Check sheet for the modelled part. Datum: model origin and axes. Units: mm. Face numbers are marked on the shaded views. A direction names the side the tool comes from. Round coordinates to 2 decimals unless told otherwise and drop trailing zeros. Order: outer loops, then holes, each group sorted by start corner. A loop starts at its lowest first (then second) coordinate and runs counter-clockwise, first axis right, second up. Notation, with made-up numbers: (38.5, -19.5) -> (49.5, -19.5) arc R17 ccw to (49.5, -8.5) -> close; hole circle Ø5 at (17, 22.5). An arc over 180 degrees is marked (long way). Answer in a Markdown table with one row per item.
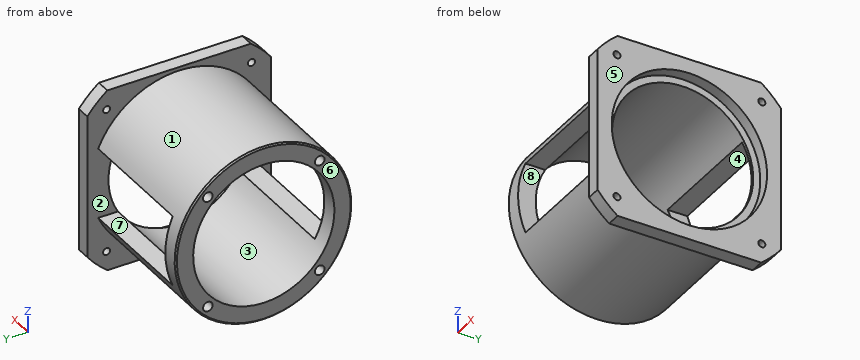
```python
from build123d import *

# Parameters (mm, degrees)
SKETCH_1_R               = 62.5
EXTRUDE_1_DEPTH          = 100
SKETCH_2_R               = 82.5
EXTRUDE_2_DEPTH          = 10
SKETCH_3_OUTSIDE_W       = 218.594
SKETCH_3_OUTSIDE_H       = 218.594
SKETCH_3_OUTSIDE_W_2     = 130
SKETCH_3_OUTSIDE_H_2     = 130
CUT_EXTRUDE_1_DEPTH      = 161.351177108
SKETCH_4_R               = 55
CUT_EXTRUDE_2_DEPTH      = 8
PATTERN_CIRCULAR_1_COUNT = 4
SKETCH_7_R               = 50
CUT_EXTRUDE_3_DEPTH      = 138.309868546
CUT_EXTRUDE_4_DEPTH      = 144.352711868
CUT_EXTRUDE_4_DEPTH_BACK = 144.352711868
SKETCH_8_W               = 88
SKETCH_8_H               = 50
PATTERN_CIRCULAR_2_COUNT = 4
CHAMFER_1_SIZE           = 1


with BuildPart() as part:
    # 草图1 → 凸台-拉伸1 (new body)
    with BuildSketch(Plane(origin=(0, 0, 0), x_dir=(0, 0, -1), z_dir=(1, 0, 0))):
        Circle(SKETCH_1_R)
    extrude(amount=EXTRUDE_1_DEPTH)

    # 草图2 → 凸台-拉伸2 (add)
    with BuildSketch(Plane(origin=(100, 0, 0), x_dir=(0, 0, -1), z_dir=(1, 0, 0))):
        Circle(SKETCH_2_R)
    extrude(amount=EXTRUDE_2_DEPTH)

    # 草图3 outside → 切除-拉伸1 (cut, through all)
    with BuildSketch(Plane(origin=(110, 0, 0), x_dir=(0, 0, -1), z_dir=(1, 0, 0))):
        Rectangle(SKETCH_3_OUTSIDE_W, SKETCH_3_OUTSIDE_H)
        Rectangle(SKETCH_3_OUTSIDE_W_2, SKETCH_3_OUTSIDE_H_2, mode=Mode.SUBTRACT)
    extrude(amount=-CUT_EXTRUDE_1_DEPTH, mode=Mode.SUBTRACT)

    # 草图4 → 切除-拉伸2 (cut)
    with BuildSketch(Plane(origin=(110, 0, 0), x_dir=(0, 0, -1), z_dir=(1, 0, 0))):
        Circle(SKETCH_4_R)
    extrude(amount=-CUT_EXTRUDE_2_DEPTH, mode=Mode.SUBTRACT)

    # 草图6 → M6 螺纹孔1 (revolve, cut)
    with BuildSketch(Plane(origin=(110, 51.265241636, 51.265241636), x_dir=(0, 0, -1), z_dir=(0, 1, 0))):
        Polygon((0, 0), (0, 16.502151548), (2.5, 15), (2.5, 0), align=None)
    hole_wizard_m6_1 = revolve(axis=Axis((116.35, 51.265241636, 51.265241636), (-1, 0, 0)), mode=Mode.SUBTRACT)

    # 阵列(圆周)1: M6 螺纹孔1 ×4 about axis
    pattern_circular_1_axis = Axis((0, 0, 0), (1, 0, 0))
    for i in range(1, PATTERN_CIRCULAR_1_COUNT):
        add(hole_wizard_m6_1.rotate(pattern_circular_1_axis, i * 360 / PATTERN_CIRCULAR_1_COUNT), mode=Mode.SUBTRACT)

    # 草图7 → 切除-拉伸3 (cut, through all)
    with BuildSketch(Plane(origin=(102, 0, 0), x_dir=(0, 0, -1), z_dir=(1, 0, 0))):
        Circle(SKETCH_7_R)
    extrude(amount=-CUT_EXTRUDE_3_DEPTH, mode=Mode.SUBTRACT)

    # 草图8 → 切除-拉伸4 (cut, two sides: drawn at the far end of the back side and taken through both)
    with BuildSketch(Plane(origin=(0, 0, 0), x_dir=(1, 0, 0), z_dir=(0, 1, 0)).offset(-CUT_EXTRUDE_4_DEPTH_BACK)):
        with Locations((56, 0)):
            Rectangle(SKETCH_8_W, SKETCH_8_H)
    extrude(amount=CUT_EXTRUDE_4_DEPTH + CUT_EXTRUDE_4_DEPTH_BACK, mode=Mode.SUBTRACT)

    # 草图10 → M8 螺纹孔1 (revolve, cut)
    with BuildSketch(Plane(origin=(0, 39.597979746, -39.597979746), x_dir=(0, 0, 1), z_dir=(0, 1, 0))):
        Polygon((0, 0), (0, 21.792926105), (3.4, 19.75), (3.4, 0), align=None)
    hole_wizard_m8_1 = revolve(axis=Axis((-6.35, 39.597979746, -39.597979746), (1, 0, 0)), mode=Mode.SUBTRACT)

    # 阵列(圆周)2: M8 螺纹孔1 ×4 about axis
    pattern_circular_2_axis = Axis((0, 0, 0), (1, 0, 0))
    for i in range(1, PATTERN_CIRCULAR_2_COUNT):
        add(hole_wizard_m8_1.rotate(pattern_circular_2_axis, i * 360 / PATTERN_CIRCULAR_2_COUNT), mode=Mode.SUBTRACT)

    # 倒角1
    chamfer_1_edges = [part.edges().sort_by_distance(p)[0] for p in [
        (0, 0, 62.5),
    ]]
    chamfer(chamfer_1_edges, length=CHAMFER_1_SIZE)


solid = part.part
```
(1) Tool access check on the marked faces 1, 2, 3 and 4. Record the directions out of +Z, -Z, +X, -X, +Y, -Y that give a thin tool (end or side, any length) a straight path to the whole face; none if there is none.
Solutions:
| item | result |
|---|---|
| face 1 | -X |
| face 2 | none |
| face 3 | +X, -X |
| face 4 | +Y, -Y |
(2) Draft check along X on the marked faces 5, 6, 7 and 8. Enter one of: pulls with the +X half, pulls with the -X half, needs draft (parallel to the pull), parting line crosses it, or undercut.
Solutions:
| item | result |
|---|---|
| face 5 | pulls with the +X half |
| face 6 | pulls with the -X half |
| face 7 | undercut |
| face 8 | undercut |
(3) Section check A-A on x = 50. Record the boundary of the cut face in (y, z), plus the area to 3 significant figures.
Solutions:
| item | result |
|---|---|
| outline | (-57.28, -25) arc R62.5 ccw to (57.28, -25) -> (43.3, -25) arc R50 cw to (-43.3, -25) -> close; (-57.28, 25) -> (-43.3, 25) arc R50 cw to (43.3, 25) -> (57.28, 25) arc R62.5 ccw to start |
| area | 3,120 mm^2 |
(4) Scan lines: probe 1 along Y at (x, z) = (103.5, -21); probe 2 along Z at (x, y) = (43.5, 31); probe 3 along Z at (x, y) = (17.5, -35.5). Record each from-to range of solid material in increasing order. Write a range as from..to.
Solutions:
| item | result |
|---|---|
| probe 1 | -65..-50.83, 50.83..65 |
| probe 2 | -54.27..-39.23, 39.23..54.27 |
| probe 3 | -51.44..-35.21, 35.21..51.44 |
(5) Section check B-B on y = 0. Record the boundary of the cut face in (x, z), plus the area to 3 significant figures.
Solutions:
| item | result |
|---|---|
| outline | (0, -61.5) -> (1, -62.5) -> (100, -62.5) -> (100, -65) -> (110, -65) -> (110, -55) -> (102, -55) -> (102, -50) -> (0, -50) -> close; (0, 50) -> (102, 50) -> (102, 55) -> (110, 55) -> (110, 65) -> (100, 65) -> (100, 62.5) -> (1, 62.5) -> (0, 61.5) -> close |
| area | 2,720 mm^2 |
(6) Depth check by flat-ended pin: pin 1 Ø6.5 at (y, z) = (-51.27, 51.27) entering from -X; pin 2 Ø6 at (y, z) = (-39.6, 39.6) entering from -X; pin 3 Ø4 at (x, y) = (51, 51) entering from +Z; pin 4 Ø3 at (x, z) = (14, 18) entering from +Y. Enter the tip coordinate at first touch or a pass-through.
Solutions:
| item | result |
|---|---|
| pin 1 | x = 100 |
| pin 2 | x = 19.99 |
| pin 3 | z = 38.8 |
| pin 4 | through |
(7) Section check C-C on z = 0. Record the boundary of the cut face in (x, y).
Solutions:
| item | result |
|---|---|
| outline | (0, -61.5) -> (1, -62.5) -> (12, -62.5) -> (12, -50) -> (0, -50) -> close; (0, 50) -> (12, 50) -> (12, 62.5) -> (1, 62.5) -> (0, 61.5) -> close; (100, -65) -> (110, -65) -> (110, -55) -> (102, -55) -> (102, -50) -> (100, -50) -> close; (100, 50) -> (102, 50) -> (102, 55) -> (110, 55) -> (110, 65) -> (100, 65) -> close |
